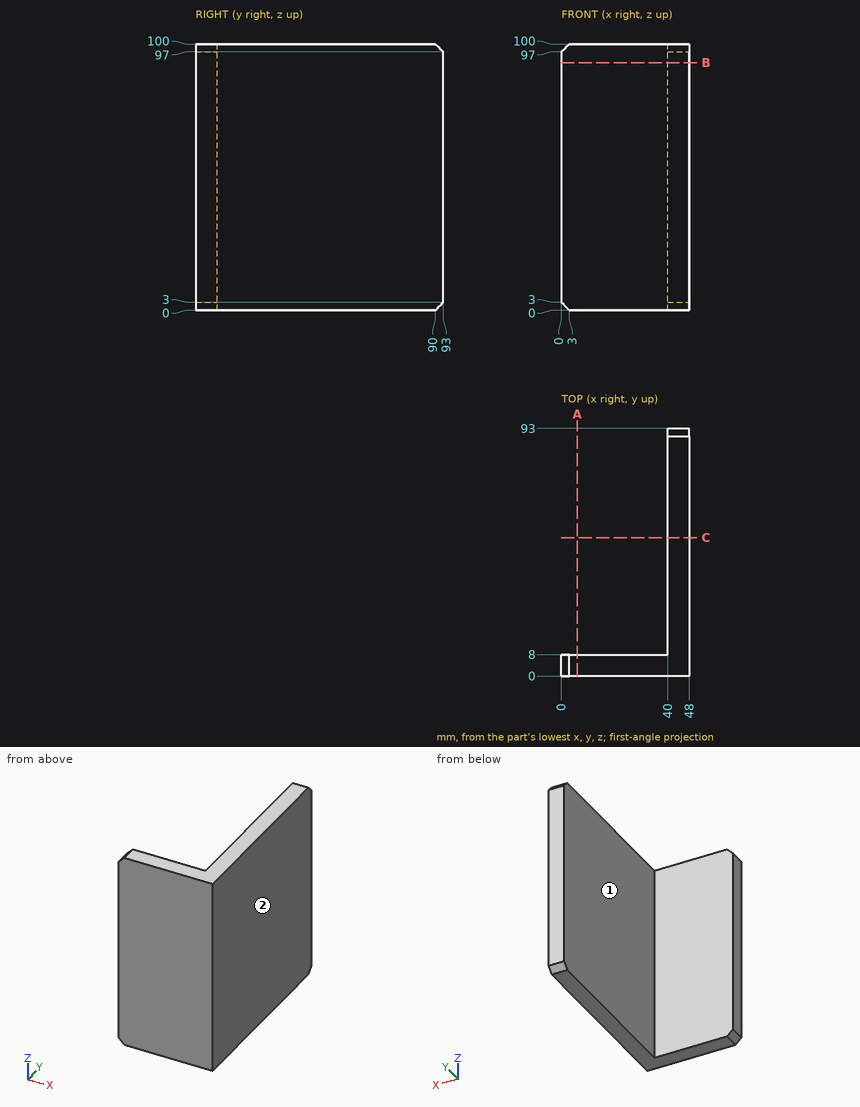
Check sheet for the drawn part. Datum: minimum x, y, z corner. Units: mm. A direction names the side the tool comes from. Give positions to 0.01 mm unless a question says otherwise; leave off trailing zeros. Loops run counter-clockwise (first coordinate to the right, second up) from the corner with the lowest first, then second, coordinate; pieces in that order, holes last.
1) Sectioned sample at C-C, the plane y = 52. Enter the section's corners in (x, z).
2) Sectioned sample at B-B, the plane z = 93. Enter the section's corners in (x, y), then the cut area to 3 significant figures.
3) Thickness scan on line 1 along Y through (x, z) = (30, 89.5); line 2 along X through (y, z) = (9.5, 58). Record the ranges inside material, lowest first.
4) Set-up check for the marked faces 1 and 2: record each of +Z, -Z, +X, -X, +Y, -Y from which the full face is reachable in a straight line by a thin tool's end or side.
5) Sectioned sample at A-A, the plane x = 6. Enter the section's corners in (y, z).
6) Depth check by flat-ended pin: pin 1 Ø1.5 at (y, z) = (69, 81.5) entering from -X; pin 2 Ø2 at (x, z) = (29.5, 57) entering from +Y. Enter the tip coordinate at first touch or a pass-through.
Answers:
1. outline: (40, 0) - (48, 0) - (48, 100) - (40, 100) - close
2. outline: (0, 0) - (48, 0) - (48, 93) - (40, 93) - (40, 8) - (0, 8) - close
2. area: 1,060 mm2
3. line 1: y = 0 to 8
3. line 2: x = 40 to 48
4. face 1: +Z, -Z, -X, +Y
4. face 2: +Z, -Z, +X, +Y, -Y
5. outline: (0, 0) - (8, 0) - (8, 100) - (0, 100) - close
6. pin 1: stops at x = 40
6. pin 2: stops at y = 8
